from build123d import *

# Parameters (mm, degrees)
SKETCH1_R           = 5
BOSS_EXTRUDE1_DEPTH = 20
SKETCH2_R           = 3
BOSS_EXTRUDE2_DEPTH = 15
CHAMFER1_SIZE       = 0.5


with BuildPart() as part:
    # Sketch1 → Boss-Extrude1 (new body)
    with BuildSketch(Plane(origin=(0, 0, 0), x_dir=(1, 0, 0), z_dir=(0, 1, 0))):
        with Locations(Location((0, 0, 0), (0, 0, 270))):
            Circle(SKETCH1_R)
    extrude(amount=BOSS_EXTRUDE1_DEPTH)

    # Sketch2 → Boss-Extrude2 (add)
    with BuildSketch(Plane.XZ):
        with Locations(Location((0, 0, 0), (0, 0, 270))):
            Circle(SKETCH2_R)
    extrude(amount=BOSS_EXTRUDE2_DEPTH)

    # Chamfer1
    chamfer1_edges = [part.edges().sort_by_distance(p)[0] for p in [
        (0, 0, -5),
        (0, 20, -5),
        (0, -15, 3),
    ]]
    chamfer(chamfer1_edges, length=CHAMFER1_SIZE)


solid = part.part
Read the model definition and answer for the solid it produces. Units are mm, in the model's axes. A direction names the side the tool comes from. Coordinates: 2 decimals unless noted, no trailing zeros. Order: outer loops, then holes, each group sorted by start corner. A loop starts at its lowest first (then second) coordinate and runs counter-clockwise, first axis right, second up. Notation, with made-up numbers: (16.25, -34) -> (63.25, -34) arc R31 ccw to (63.25, -7) -> close; hole circle Ø7 at (86, 27.5). An arc over 180 degrees is marked (long way). Answer as a JSON object with one key per item and string values.
1) A tool of negligible diameter and unlimited length cuts with its end or side. For faces 1 (the face through (0, 20, 0)), 2 (the face through (-3, 0, 1)), from which of +Z, -Z, +X, -X, +Y, -Y can it reach the whole face along a straight path? Write none if from no direction.
Model answer:
{"face 1": "+Z, -Z, +X, -X, +Y", "face 2": "-Y"}
2) A cutting plane is placed at C-C, the plane y = -3.5. Determine the outline of the cut face in (x, z).
Model answer:
{"outline": "circle Ø6 at (0, 0)"}
3) A cutting plane is placed at D-D, the plane y = 5. Determine the outline of the cut face in (x, z).
Model answer:
{"outline": "circle Ø10 at (0, 0)"}
4) A cutting plane is placed at A-A, the plane x = 0. Determine the outline of the cut face in (y, z).
Model answer:
{"outline": "(-15, -2.5) -> (-14.5, -3) -> (0, -3) -> (0, -4.5) -> (0.5, -5) -> (19.5, -5) -> (20, -4.5) -> (20, 4.5) -> (19.5, 5) -> (0.5, 5) -> (0, 4.5) -> (0, 3) -> (-14.5, 3) -> (-15, 2.5) -> close"}
5) Consider line 1 along Y through (x, z) = (-3.5, -2.5); line 2 along X through (y, z) = (6, -0.25). Determine where each line is inside the solid, lowest interval first. Write a range as from..to.
Model answer:
{"line 1": "y = 0..20", "line 2": "x = -4.99..4.99"}
6) Each of these flat-tipped pins is pushed along its axis until it touches: pin 1 (1 mm diameter, centred on x = 3.5, z = 2.5, fed in from -Y); pin 2 (3 mm diameter, centred on y = -10, z = 3.5, fed in from -X); pin 3 (5 mm diameter, centred on y = -7.5, z = 0.5, fed in from +X). Where does it stop, or does it pass through?
Model answer:
{"pin 1": "stops at y = 0", "pin 2": "stops at x = -2.24", "pin 3": "stops at x = 3"}
7) A cutting plane is placed at B-B, the plane z = 0. Determine the outline of the cut face in (x, y).
Model answer:
{"outline": "(-5, 0.5) -> (-4.5, 0) -> (-3, 0) -> (-3, -14.5) -> (-2.5, -15) -> (2.5, -15) -> (3, -14.5) -> (3, 0) -> (4.5, 0) -> (5, 0.5) -> (5, 19.5) -> (4.5, 20) -> (-4.5, 20) -> (-5, 19.5) -> close"}
